Check sheet for the modelled part. Datum: model origin and axes. Units: mm. A direction names the side the tool comes from. Give positions to 0.01 mm unless a question says otherwise; leave off trailing zeros. Order: outer loops, then holes, each group sorted by start corner. A loop starts at its lowest first (then second) coordinate and runs counter-clockwise, first axis right, second up.
```python
from build123d import *

# Parameters (mm, degrees)
SKETCH1_W                      = 415
SKETCH1_H                      = 70
BOSS_EXTRUDE1_DEPTH            = 15
SKETCH2_R                      = 3.4
SKETCH2_R_2                    = 12
CUT_EXTRUDE1_DEPTH             = 211.965044498
SKETCH10_W                     = 15
SKETCH10_H                     = 60
CUT_EXTRUDE2_DEPTH             = 211.965044498
F_6_8_6_8_DIAMETER_HOLE1_D     = 6.8
F_6_8_6_8_DIAMETER_HOLE1_DEPTH = 12.4
F_6_8_6_8_DIAMETER_HOLE1_TIP   = 2.042926105
FILLET1_R                      = 5
FILLET2_R                      = 5
M6_TAPPED_HOLE1_D              = 5
M6_TAPPED_HOLE1_DEPTH          = 15
M6_TAPPED_HOLE1_TIP            = 1.502151548


with BuildPart() as part:
    # Sketch1 → Boss-Extrude1 (new body)
    with BuildSketch(Plane.XY):
        Rectangle(SKETCH1_W, SKETCH1_H)
    extrude(amount=BOSS_EXTRUDE1_DEPTH)

    # Sketch2 → Cut-Extrude1 (cut, through all)
    with BuildSketch(Plane.XY.offset(15)):
        with Locations((-182.5, 5)):
            Circle(SKETCH2_R)
        with Locations((-142.5, 5)):
            Circle(SKETCH2_R_2)
        with Locations((142.5, 5)):
            Circle(SKETCH2_R_2)
        with Locations((182.5, 5)):
            Circle(SKETCH2_R)
    extrude(amount=-CUT_EXTRUDE1_DEPTH, mode=Mode.SUBTRACT)

    # Sketch10 → Cut-Extrude2 (cut, through all)
    with BuildSketch(Plane.XY.offset(15)):
        with Locations((-200, 5)):
            Rectangle(SKETCH10_W, SKETCH10_H)
        with Locations((200, 5)):
            Rectangle(SKETCH10_W, SKETCH10_H)
    extrude(amount=-CUT_EXTRUDE2_DEPTH, mode=Mode.SUBTRACT)

    # Ø6.8 (6.8) Diameter Hole1
    with Locations(Plane(origin=(0, -35, 0), x_dir=(-1, 0, 0), z_dir=(0, -1, 0))):
        with Locations((-202.5, -7.5), (202.5, -7.5)):
            Hole(F_6_8_6_8_DIAMETER_HOLE1_D / 2, depth=F_6_8_6_8_DIAMETER_HOLE1_DEPTH)
            with Locations((0, 0, -(F_6_8_6_8_DIAMETER_HOLE1_DEPTH + F_6_8_6_8_DIAMETER_HOLE1_TIP / 2))):  # 118° drill point
                Cone(0, F_6_8_6_8_DIAMETER_HOLE1_D / 2, F_6_8_6_8_DIAMETER_HOLE1_TIP, mode=Mode.SUBTRACT)

    # Fillet1
    fillet1_edges = [part.edges().sort_by_distance(p)[0] for p in [
        (-192.5, -25, 7.5),
        (192.5, -25, 7.5),
    ]]
    fillet(fillet1_edges, radius=FILLET1_R)

    # Fillet2
    fillet2_edges = [part.edges().sort_by_distance(p)[0] for p in [
        (-192.5, 35, 7.5),
        (192.5, 35, 7.5),
    ]]
    fillet(fillet2_edges, radius=FILLET2_R)

    # M6 Tapped Hole1
    with Locations(Plane(origin=(0, -35, 0), x_dir=(-1, 0, 0), z_dir=(0, -1, 0))):
        with Locations((125, -7.5), (-125, -7.5)):
            Hole(M6_TAPPED_HOLE1_D / 2, depth=M6_TAPPED_HOLE1_DEPTH)
            with Locations((0, 0, -(M6_TAPPED_HOLE1_DEPTH + M6_TAPPED_HOLE1_TIP / 2))):  # 118° drill point
                Cone(0, M6_TAPPED_HOLE1_D / 2, M6_TAPPED_HOLE1_TIP, mode=Mode.SUBTRACT)


solid = part.part
```
(1) Sectioned sample at B-B (x = 202.5). Enter the section's corners in (y, z), plus the area to 3 significant figures.
(2) Sectioned sample at A-A (x = -142.5). Enter the section's corners in (y, z), plus the area to 3 significant figures.
(3) Tool access check on faces 5 (the face through (-3, -35, 7)), 6 (the face through (201, -25, 11)), 7 (the face through (-204, -25, 11)). Record the directions out of +Z, -Z, +X, -X, +Y, -Y that give a thin tool (end or side, any length) a straight path to the whole face; none if there is none.
(4) Release check for a two-part mould opening along Z. For faces 1 (the face through (-3, 0, 0)), 2 (the face through (-205.9, -29.9, 7.4)), 3 (the face through (199.1, -29.9, 7.4)), 4 (the face through (179.1, 5.1, 7.6)) record: released by +Z, released by -Z, zero draft, split by the parting line, or undercut.
(5) Go/stop test with flat-tipped pins: P1, Ø10, axis at x = 104.5, y = -25, coming from the -Z side; P2, Ø8, axis at x = 202.5, z = 7.5, coming from the +Y side; P3, Ø4.5, axis at y = -5.5, z = 9.5, coming from the -X side; P4, Ø3, axis at y = -8.5, z = 11, coming from the +X side. Record where each tip stops, or that it passes through.
(6) Thickness scan on L1, parallel to Y at x = 182.5, z = 5; L2, parallel to Y at x = 142.5, z = 7; L3, parallel to Z at x = -125, y = -29.25. Record the ranges inside material, lowest first.
Values follow:
1. outline: (-35, 0) - (-25, 0) - (-25, 4.1) - (-35, 4.1) - close; (-35, 10.9) - (-25, 10.9) - (-25, 15) - (-35, 15) - close
1. area: 82.0 mm2
2. outline: (-35, 0) - (-7, 0) - (-7, 15) - (-35, 15) - close; (17, 0) - (35, 0) - (35, 15) - (17, 15) - close
2. area: 690 mm2
3. face 5: +Z, -Z, +X, -X, -Y
3. face 6: +Z, -Z, +X, +Y
3. face 7: +Z, -Z, -X, +Y
4. face 1: released by -Z
4. face 2: undercut
4. face 3: undercut
4. face 4: zero draft
5. P1: stops at z = 0
5. P2: stops at y = -25
5. P3: stops at x = -192.5
5. P4: stops at x = 192.5
6. L1: y = -35 to 1.6, 8.4 to 35
6. L2: y = -35 to -7, 17 to 35
6. L3: z = 0 to 5, 10 to 15
